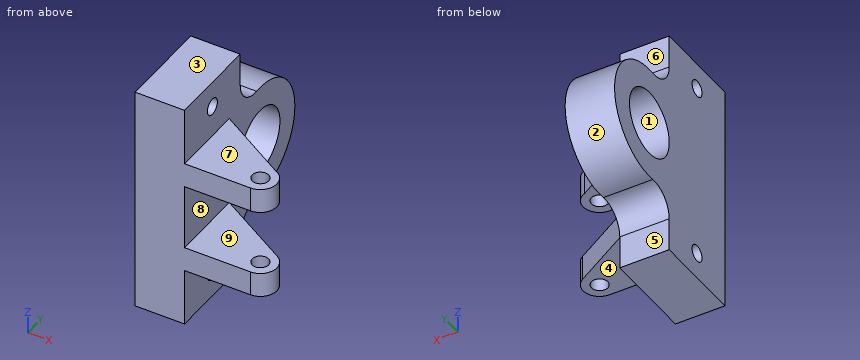
from build123d import *

# Parameters (mm, degrees)
PILLOW_BLOCK_BASE_DEPTH = 15
LUG_ARM_1_DEPTH         = 15
LUG_START               = -15
LUG_ARM_2_DEPTH         = 15
LUG_PIN_HOLE_SKETCH_R   = 5
LUG_PIN_HOLE_DEPTH      = 100
MOUNTING_HOLES_SKETCH_R = 5
MOUNTING_HOLES_2X_DEPTH = 100
SHAFT_BORE_SKETCH_R     = 20
SHAFT_BORE_DEPTH        = 100


with BuildPart() as part:
    # Base Profile Sketch → Pillow Block Base (new, symmetric)
    with BuildSketch(Plane(origin=(0, 0, 0), x_dir=(0, 0, -1), z_dir=(1, 0, 0))):
        with BuildLine():
            Line((0, 0), (-70, 0))
            Line((-70, 0), (-70, 56))
            Line((-70, 56), (-49.749371855, 56))
            ThreePointArc((-49.749371855, 56), (-38.625074125, 60.937694101), (-34.824560299, 72.5))
            ThreePointArc((-34.824560299, 72.5), (0, 111), (34.824560299, 72.5))
            ThreePointArc((34.824560299, 72.5), (38.625074125, 60.937694101), (49.749371855, 56))
            Line((49.749371855, 56), (70, 56))
            Line((70, 56), (70, 0))
            Line((70, 0), (0, 0))
        make_face()
    extrude(amount=PILLOW_BLOCK_BASE_DEPTH, both=True)

    # Lug Arm 1 Sketch → Lug Arm 1 (add)
    with BuildSketch(Plane.XY.offset(20)):
        with BuildLine():
            Line((15, 0), (55, 0))
            ThreePointArc((55, 0), (64.845332755, 8.248023132), (58.449759048, 19.386115411))
            Line((58.449759048, 19.386115411), (15, 45))
            Line((15, 45), (15, 0))
        make_face()
    extrude(amount=LUG_ARM_1_DEPTH)

    # Lug Arm 2 Sketch → Lug Arm 2 (add)
    with BuildSketch(Plane.XY.offset(-20).offset(LUG_START)):
        with BuildLine():
            Line((15, 0), (55, 0))
            ThreePointArc((55, 0), (64.651503897, 7.383041358), (60.051517306, 18.630305493))
            Line((60.051517306, 18.630305493), (15, 45))
            Line((15, 45), (15, 0))
        make_face()
    extrude(amount=LUG_ARM_2_DEPTH)

    # Lug Pin Hole Sketch → Lug Pin Hole (cut)
    with BuildSketch(Plane(origin=(0, 0, -35), x_dir=(-1, 0, 0), z_dir=(0, 0, -1))):
        with Locations((-55, 10)):
            Circle(LUG_PIN_HOLE_SKETCH_R)
    extrude(amount=-LUG_PIN_HOLE_DEPTH, mode=Mode.SUBTRACT)

    # Mounting Holes Sketch → Mounting Holes 2x (cut)
    with BuildSketch(Plane(origin=(15, 0, 0), x_dir=(0, 0, -1), z_dir=(1, 0, 0))):
        with Locations((-54, 28)):
            Circle(MOUNTING_HOLES_SKETCH_R)
        with Locations((54, 28)):
            Circle(MOUNTING_HOLES_SKETCH_R)
    extrude(amount=-MOUNTING_HOLES_2X_DEPTH, mode=Mode.SUBTRACT)

    # Shaft Bore Sketch → Shaft Bore (cut)
    with BuildSketch(Plane(origin=(15, 0, 0), x_dir=(0, 0, -1), z_dir=(1, 0, 0))):
        with Locations((0, 76)):
            Circle(SHAFT_BORE_SKETCH_R)
    extrude(amount=-SHAFT_BORE_DEPTH, mode=Mode.SUBTRACT)


solid = part.part
Could you check a few things on this model? Use its own coordinates, in mm. Face numbers are marked on the shaded views. A direction names the side the tool comes from. Coordinates: 2 decimals unless noted, no trailing zeros. Order: outer loops, then holes, each group sorted by start corner. A loop starts at its lowest first (then second) coordinate and runs counter-clockwise, first axis right, second up.
Q1. Suppose I cut it at A-A on z = 54. Please give me the cut outline in (x, y), and give its area (3 significant figures).
Q2. Please list where these lines run through material, in increasing order: L1, parallel to Y at x = -0.75, z = -54; L2, parallel to X at y = 31.5, z = -1; L3, parallel to Y at x = 55, z = 28.5.
Q3. Will these pins go through, and if not, where does the flat tip stop? pin 1 (6 mm diameter, centred on x = 38, y = 34, fed in from -Z); pin 2 (11.5 mm diameter, centred on y = 28, z = -54, fed in from -X); pin 3 (2 mm diameter, centred on x = -5.5, z = -17, fed in from +Y); pin 4 (13 mm diameter, centred on x = 55, y = 10, fed in from +Z).
Q4. Thinking about a two-plate mould opening in Z: for the marked faces 1, 2, 3 and 4, which applies, released by +Z, released by -Z, zero draft, split by the parting line, or undercut?
Q5. Suppose I cut it at D-D on y = 76. Please give me the cut outline in (x, z), and give its area (3 significant figures).
Q6. Which directions (+Z, -Z, +X, -X, +Y, -Y) give clear straight access to the entire face, cutting with the end or side of a thin tool? Please do the marked faces 5, 6, 7, 8 and 9.
Q7. Suppose I cut it at C-C on x = 52. Please give me the cut outline in (y, z).
Q8. Suppose I cut it at B-B on y = 10. Please give me the cut outline in (x, z), and give its area (3 significant figures).
Answer:
1. outline: (-15, 0) - (15, 0) - (15, 23) - (-15, 23) - close; (-15, 33) - (15, 33) - (15, 56) - (-15, 56) - close
1. area: 1,380 mm2
2. L1: y = 0 to 23, 33 to 56
2. L2: x = -15 to 15
2. L3: y = 0 to 5, 15 to 21.42
3. pin 1: stops at z = -35
3. pin 2: stops at x = -15
3. pin 3: stops at y = 107.13
3. pin 4: stops at z = 35
4. face 1: undercut
4. face 2: split by the parting line
4. face 3: released by +Z
4. face 4: released by -Z
5. outline: (-15, -35) - (15, -35) - (15, -20) - (-15, -20) - close; (-15, 20) - (15, 20) - (15, 35) - (-15, 35) - close
5. area: 900 mm2
6. face 5: -Z, +X, -X, +Y
6. face 6: +Z, +X, -X, +Y
6. face 7: +Z, +X, +Y, -Y
6. face 8: +X, +Y
6. face 9: +X, +Y, -Y
7. outline: (0, -35) - (6, -35) - (6, -20) - (0, -20) - close; (0, 20) - (6, 20) - (6, 35) - (0, 35) - close; (14, -35) - (23.34, -35) - (23.34, -20) - (14, -20) - close; (14, 20) - (23.19, 20) - (23.19, 35) - (14, 35) - close
8. outline: (-15, -70) - (15, -70) - (15, -35) - (50, -35) - (50, -20) - (15, -20) - (15, 20) - (50, 20) - (50, 35) - (15, 35) - (15, 70) - (-15, 70) - close; (60, -35) - (65, -35) - (65, -20) - (60, -20) - close; (60, 20) - (65, 20) - (65, 35) - (60, 35) - close
8. area: 5,400 mm2
